Work out the finished part from the listing and answer in its coordinate system (mm). Give positions to 0.01 mm unless a question says otherwise; leave off trailing zeros. Order: outer loops, then holes, each group sorted by start corner. A loop starts at its lowest first (then second) coordinate and runs counter-clockwise, first axis right, second up. Notation, with made-up numbers: (-24, -5) - (23, -5) arc R20 cw to (23, 8) - close; hole circle Ø2 at (-31.75, 82.25). An arc over 180 degrees is marked (long way). Return JSON: item names as keys, results as strings. Group by question number.
from build123d import *

# Parameters (mm, degrees)
WIRE_SWEEP_4_PROFILE_R = 2


with BuildPart() as part:
    # Wire Sweep Ø4: sweep along a path in Clip Wire Path
    with BuildLine(Plane.XY) as wire_sweep_4_path:
        Line((0, 0), (-68, 0))
        ThreePointArc((-68, 0), (-80.5, 12.5), (-68, 25))
        ThreePointArc((-68, 25), (-62.93740019, 23.928914347), (-58.742396863, 20.899213306))
        Line((-58.742396863, 20.899213306), (-46.259260276, 7.140314678))
        ThreePointArc((-46.259260276, 7.140314678), (-43.2855546, 5.553479039), (-39.980410457, 6.214535003))
        Line((-39.980410457, 6.214535003), (-33.8729527, 9.885464997))
        ThreePointArc((-33.8729527, 9.885464997), (-31.656450173, 10.587073207), (-29.362263704, 10.210448754))
        Line((-29.362263704, 10.210448754), (-16.862956001, 4.964827953))
        ThreePointArc((-16.862956001, 4.964827953), (-14.811169509, 4.576643597), (-12.779773841, 5.060323807))
        Line((-12.779773841, 5.060323807), (-4.5, 9))
    # Wire Sweep Ø4 profile (on start of the path) → Wire Sweep Ø4 (sweep)
    with BuildSketch(Plane(origin=(0, 0, 0), x_dir=(0, -1, 0), z_dir=(-1, 0, 0))):
        Circle(WIRE_SWEEP_4_PROFILE_R)
    sweep(path=wire_sweep_4_path.line)


solid = part.part
1. Consider probe 1 along X at (y, z) = (10, 0.7); probe 2 along X at (y, z) = (12.5, -1); probe 3 along Y at (x, z) = (-17, 1.1). Determine where each line is inside the solid, lowest interval first. Write a range as from..to.
2. Determine the mould class of faces 1 (the flat face through (-4.5, 9, 0)), 2 (the cylindrical face through (-34, 0, -2)), 3 (the cylindrical face through (-23.64, 6.09, -1.22)) for opening direction X: released by +X, released by -X, zero draft, split by the parting line, or undercut.
3. Each of these flat-tipped pins is pushed along its axis until it touches: pin 1 (1 mm diameter, centred on x = -22.5, z = 1, fed in from -Y); pin 2 (1.5 mm diameter, centred on y = 21, z = -1.5, fed in from +X); pin 3 (2 mm diameter, centred on x = -50, y = 6.5, fed in from +Z). Where does it stop, or does it pass through?
4. The part is cut by section A-A (z = -0.8). Give the vertices of the cut face in (x, y).
Answers:
{
 "1": {"probe 1": "x = -82.15..-78.33, -51.38..-46.32, -37.32..-24.02, -6.76..-4.98", "probe 2": "x = -82.23..-78.77, -53.46..-48.78", "probe 3": "y = -1.67..1.67, 3.23..6.83"},
 "2": {"face 1": "released by +X", "face 2": "zero draft", "face 3": "undercut"},
 "3": {"pin 1": "stops at y = -1.94", "pin 2": "stops at x = -55.99", "pin 3": "passes through"},
 "4": {"outline": "(-68, -1.83) - (0, -1.83) - (0, 1.83) - (-68, 1.83) arc R10.67 cw (long way) to (-60.1, 19.67) - (-47.62, 5.91) arc R6.83 ccw to (-39.04, 4.64) - (-32.93, 8.31) arc R3.17 cw to (-30.07, 8.52) - (-17.57, 3.27) arc R6.83 ccw to (-11.99, 3.41) - (-3.71, 7.34) - (-5.29, 10.66) - (-13.57, 6.72) arc R3.17 cw to (-16.15, 6.66) - (-28.65, 11.9) arc R6.83 ccw to (-34.82, 11.46) - (-40.92, 7.79) arc R3.17 cw to (-44.9, 8.37) - (-57.38, 22.13) arc R14.33 ccw (long way) to start"}
}
